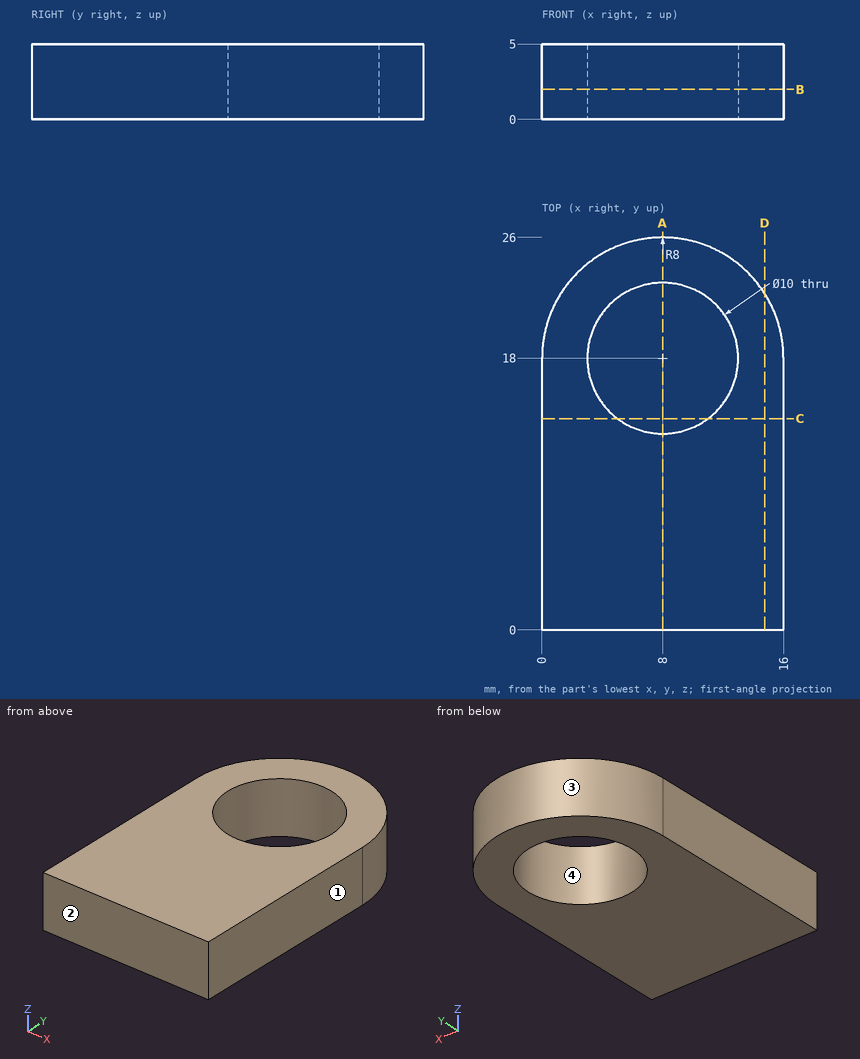
Check sheet for the drawn part. Datum: minimum x, y, z corner. Units: mm. Give positions to 0.01 mm unless a question says otherwise; leave off trailing zeros. Write each loop counter-clockwise with the first axis right and the second up, starting at its lowest first coordinate (ties: lowest second). Pieces come first, ordered by that corner, then holes. Notation, with made-up numbers: M 48,-30.75 L 81,-30.75 A5 cw 81,-26.75 Z; hole C 89.5,65.5 d9. An arc over 180 degrees is marked long. One line per question, with ' | ' between items.
1. Scan lines: line 1 along Y through (x, z) = (8, 3.2); line 2 along Y through (x, z) = (9, 2.05); line 3 along X through (y, z) = (13.5, 2). Record each from-to range of solid material in increasing order. Write a range as from..to.
Ans:
line 1: 0..13, 23..26 | line 2: 0..13.1, 22.9..25.94 | line 3: 0..5.82, 10.18..16
2. Cross-section at A-A (x = 8). Enter the section's corners in (y, z), plus the area to 3 significant figures.
Ans:
outline: M 0,0 L 13,0 L 13,5 L 0,5 Z; M 23,0 L 26,0 L 26,5 L 23,5 Z | area: 80.0 mm2
3. Cross-section at B-B (z = 2). Enter the section's corners in (x, y).
Ans:
outline: M 0,0 L 16,0 L 16,18 A8 ccw 0,18 Z; hole C 8,18 d10
4. Cross-section at D-D (x = 14.75). Enter the section's corners in (y, z), plus the area to 3 significant figures.
Ans:
outline: M 0,0 L 22.29,0 L 22.29,5 L 0,5 Z | area: 111 mm2
5. Cross-section at C-C (y = 14). Enter the section's corners in (x, z), plus the area to 3 significant figures.
Ans:
outline: M 0,0 L 5,0 L 5,5 L 0,5 Z; M 11,0 L 16,0 L 16,5 L 11,5 Z | area: 50.0 mm2
6. Mould release check, pull along Y, two halves, no side actions. Record for the marked faces 1, 2, 3 and 4: released by +Y, released by -Y, zero draft, split by the parting line, or undercut.
Ans:
face 1: zero draft | face 2: released by -Y | face 3: released by +Y | face 4: undercut
